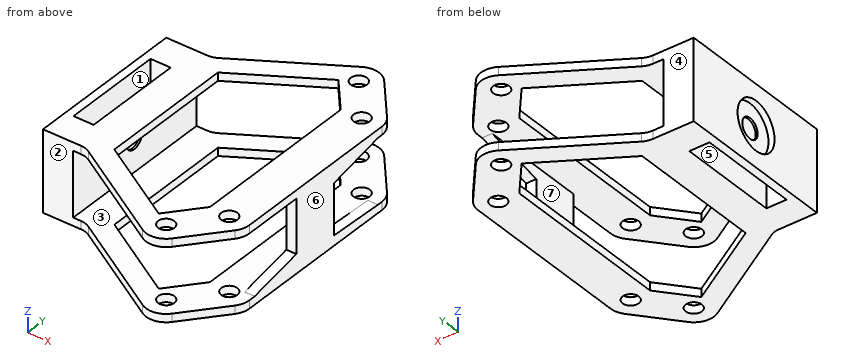
```python
from build123d import *

# Parameters (mm, degrees)
BRACKET_PROFILE_SKETCH_R    = 4
BRACKET_PROFILE_SKETCH_W    = 10
BRACKET_PROFILE_SKETCH_H    = 50
BRACKET_BODY_DEPTH          = 20
SIDE_CUTOUT_DEPTH           = 151.958708937
SIDE_CUTOUT_DEPTH_BACK      = 151.958708937
SIDE_CUTOUT_SKETCH_W        = 85
SIDE_CUTOUT_SKETCH_H        = 32
INNER_WINDOW_CUT_DEPTH      = 130.155913531
INNER_WINDOW_CUT_DEPTH_BACK = 130.155913531
INNER_WINDOW_SKETCH_W       = 32
INNER_WINDOW_SKETCH_H       = 12.117592982
INNER_WINDOW_SKETCH_H_2     = 13.000486956
SIDE_OPENINGS_CUT_DEPTH     = 40
HOLE_10_SKETCH_R            = 5
THROUGH_HOLE_10_DEPTH       = 40
RECESS_24_SKETCH_R          = 12
RECESS_24X3_DEPTH           = 3


with BuildPart() as part:
    # Bracket Profile Sketch → Bracket Body (new, symmetric)
    with BuildSketch(Plane.XY):
        with BuildLine():
            Line((18.112706939, 41.738939357), (66.624129095, 71.058341812))
            ThreePointArc((66.624129095, 71.058341812), (73.442433942, 72.363637042), (79.467576157, 68.915342115))
            Line((79.467576157, 68.915342115), (95.817576157, 49.365342115))
            ThreePointArc((95.817576157, 49.365342115), (97.546351125, 46.362517955), (98.146631916, 42.95))
            Line((98.146631916, 42.95), (98.146631916, -42.95))
            ThreePointArc((98.146631916, -42.95), (97.546351125, -46.362517955), (95.817576157, -49.365342115))
            Line((95.817576157, -49.365342115), (79.467576157, -68.915342115))
            ThreePointArc((79.467576157, -68.915342115), (73.442433942, -72.363637042), (66.624129095, -71.058341812))
            Line((66.624129095, -71.058341812), (16.651884454, -40.856045382))
            ThreePointArc((16.651884454, -40.856045382), (14.412975364, -39.88899222), (11.996631916, -39.558553013))
            Line((11.996631916, -39.558553013), (-6.853368084, -39.558553013))
            Line((-6.853368084, -39.558553013), (-6.853368084, 40.441446987))
            Line((-6.853368084, 40.441446987), (13.4574544, 40.441446987))
            ThreePointArc((13.4574544, 40.441446987), (15.873797849, 40.771886195), (18.112706939, 41.738939357))
        make_face()
        with Locations((88.146631916, 42.95)):
            Circle(BRACKET_PROFILE_SKETCH_R, mode=Mode.SUBTRACT)
        with Locations((71.796631916, 62.5)):
            Circle(BRACKET_PROFILE_SKETCH_R, mode=Mode.SUBTRACT)
        with Locations(Location((88.146631916, -42.95, 0), (0, 0, 180))):
            Circle(BRACKET_PROFILE_SKETCH_R, mode=Mode.SUBTRACT)
        with Locations(Location((71.796631916, -62.5, 0), (0, 0, 180))):
            Circle(BRACKET_PROFILE_SKETCH_R, mode=Mode.SUBTRACT)
        with Locations((2.146631916, 0)):
            Rectangle(BRACKET_PROFILE_SKETCH_W, BRACKET_PROFILE_SKETCH_H, mode=Mode.SUBTRACT)
        Polygon((23.996631916, 33.610567881), (23.996631916, -33.610567881), (64.869180084, -58.31317679), (78.146631916, -42.437079952), (78.146631916, 42.437079952), (64.869180084, 58.31317679), align=None, mode=Mode.SUBTRACT)
    extrude(amount=BRACKET_BODY_DEPTH, both=True)

    # Side Cutout Sketch → Side Cutout (cut, two sides: drawn at the far end of the back side and taken through both)
    with BuildSketch(Plane(origin=(0, 40.441446987, 0), x_dir=(1, 0, 0), z_dir=(0, 1, 0)).offset(-SIDE_CUTOUT_DEPTH_BACK)):
        with Locations((50.646631916, 0)):
            Rectangle(SIDE_CUTOUT_SKETCH_W, SIDE_CUTOUT_SKETCH_H)
    extrude(amount=SIDE_CUTOUT_DEPTH + SIDE_CUTOUT_DEPTH_BACK, mode=Mode.SUBTRACT)

    # Inner Window Sketch → Inner Window Cut (cut, two sides: drawn at the far end of the back side and taken through both)
    with BuildSketch(Plane.ZY.offset(6.853368084).offset(-INNER_WINDOW_CUT_DEPTH_BACK)):
        with Locations((0, 46.500243478)):
            Rectangle(INNER_WINDOW_SKETCH_W, INNER_WINDOW_SKETCH_H)
        with Locations((0, -46.058796491)):
            Rectangle(INNER_WINDOW_SKETCH_W, INNER_WINDOW_SKETCH_H_2)
    extrude(amount=INNER_WINDOW_CUT_DEPTH + INNER_WINDOW_CUT_DEPTH_BACK, mode=Mode.SUBTRACT)

    # Side Openings Sketch → Side Openings Cut (cut)
    with BuildSketch(Plane(origin=(98.146631916, 0, 0), x_dir=(0, 0, -1), z_dir=(1, 0, 0))):
        Polygon((-16, -39.558553013), (-16, -12.5), (10.579626048, -12.5), (16, -39.558553013), align=None)
        Polygon((-16, 40.441446987), (-9.950879321, 11.757125531), (15.049120679, 11.757125531), (16, 40.441446987), align=None)
    extrude(amount=-SIDE_OPENINGS_CUT_DEPTH, mode=Mode.SUBTRACT)

    # Hole Ø10 Sketch → Through Hole Ø10 (cut)
    with BuildSketch(Plane.ZY.offset(6.853368084)):
        Circle(HOLE_10_SKETCH_R)
    extrude(amount=-THROUGH_HOLE_10_DEPTH, mode=Mode.SUBTRACT)

    # Recess Ø24 Sketch → Recess Ø24x3 (cut)
    with BuildSketch(Plane.ZY.offset(6.853368084)):
        Circle(RECESS_24_SKETCH_R)
    extrude(amount=-RECESS_24X3_DEPTH, mode=Mode.SUBTRACT)


solid = part.part
```
For this review, take the finished solid that the model builds, in its own axes (mm). Face numbers are marked on the shaded views. A direction names the side the tool comes from. Round coordinates to 2 decimals unless told otherwise and drop trailing zeros. Write each loop counter-clockwise with the first axis right and the second up, starting at its lowest first coordinate (ties: lowest second). Pieces come first, ordered by that corner, then holes. Notation, with made-up numbers: (-28.5, 85) -> (14.5, 85) arc R6 ccw to (14.5, 89) -> close; hole circle Ø5 at (42.5, 86.5). An arc over 180 degrees is marked (long way). Use one line per item in the form item = value.
Q1. Consider section A-A (x = 2.5). State the section outline as (y, z) points, then the cut area to 3 significant figures.
Resolved:
outline = (-39.56, -20) -> (-25, -20) -> (-25, 20) -> (-39.56, 20) -> close; (25, -20) -> (40.44, -20) -> (40.44, 20) -> (25, 20) -> close
area = 1,200 mm²
Q2. The part is to be moulded in two halves that separate along Y. For the marked faces 1, 2, 3 and 4, say which applies: released by +Y, released by -Y, zero draft, split by the parting line, or undercut.
Resolved:
face_1 = undercut
face_2 = released by -Y
face_3 = zero draft
face_4 = released by +Y
Q3. Consider section C-C (y = 0). State how many separate pieces and enclosed holes the cut face has, then the cut area to 3 significant figures.
Resolved:
separate_pieces = 5
enclosed_holes = 0
area = 555 mm²
Q4. Consider section D-D (x = 53.5). State the section outline as (y, z) points.
Resolved:
outline = (-63.13, -20) -> (-51.44, -20) -> (-51.44, -16) -> (-63.13, -16) -> close; (-63.13, 16) -> (-51.44, 16) -> (-51.44, 20) -> (-63.13, 20) -> close; (51.44, -20) -> (63.13, -20) -> (63.13, -16) -> (51.44, -16) -> close; (51.44, 16) -> (63.13, 16) -> (63.13, 20) -> (51.44, 20) -> close
Q5. Clearance check with flat-ended pins moving along their axes: pin 1 Ø1.5 at (x, z) = (95.5, -0.5) entering from -Y; pin 2 Ø16 at (x, z) = (8, 4) entering from +Y; pin 3 Ø10 at (x, z) = (8.5, -4.5) entering from -Y. State where each tip first meets the part, or that it passes through.
Resolved:
pin_1 = -12.5
pin_2 = 40.44
pin_3 = -39.56
Q6. To check wall thickness, follow probe 1 along X at (y, z) = (-9, -6.5); probe 2 along Z at (x, y) = (30.5, 45.5); probe 3 along X at (y, z) = (-23, -7.5). State the ranges of each line that lie inside material, in increasing order. Write a range as from..to.
Resolved:
probe_1 = -3.85..-2.85, 7.15..8.15, 93.15..98.15
probe_2 = -20..-16, 16..20
probe_3 = -6.85..-2.85, 7.15..8.15
Q7. Machinability: for the marked faces 5, 6 and 7, which of the approach directions +Z, -Z, +X, -X, +Y, -Y give a long, thin tool a straight path to every point of the face, cutting with its end or side? Answer none if there is none.
Resolved:
face_5 = +Z, -Z
face_6 = +Z, -Z, +X, +Y, -Y
face_7 = +Y, -Y
Q8. Consider section B-B (z = 0). State the section outline as (x, y) points, then the cut area to 3 significant figures.
Resolved:
outline = (-6.85, -39.56) -> (8.15, -39.56) -> (8.15, -5) -> (7.15, -5) -> (7.15, -25) -> (-2.85, -25) -> (-2.85, -5) -> (-3.85, -5) -> (-3.85, -12) -> (-6.85, -12) -> close; (-6.85, 12) -> (-3.85, 12) -> (-3.85, 5) -> (-2.85, 5) -> (-2.85, 25) -> (7.15, 25) -> (7.15, 5) -> (8.15, 5) -> (8.15, 40.44) -> (-6.85, 40.44) -> close; (93.15, -12.5) -> (98.15, -12.5) -> (98.15, 11.76) -> (93.15, 11.76) -> close
area = 729 mm²
